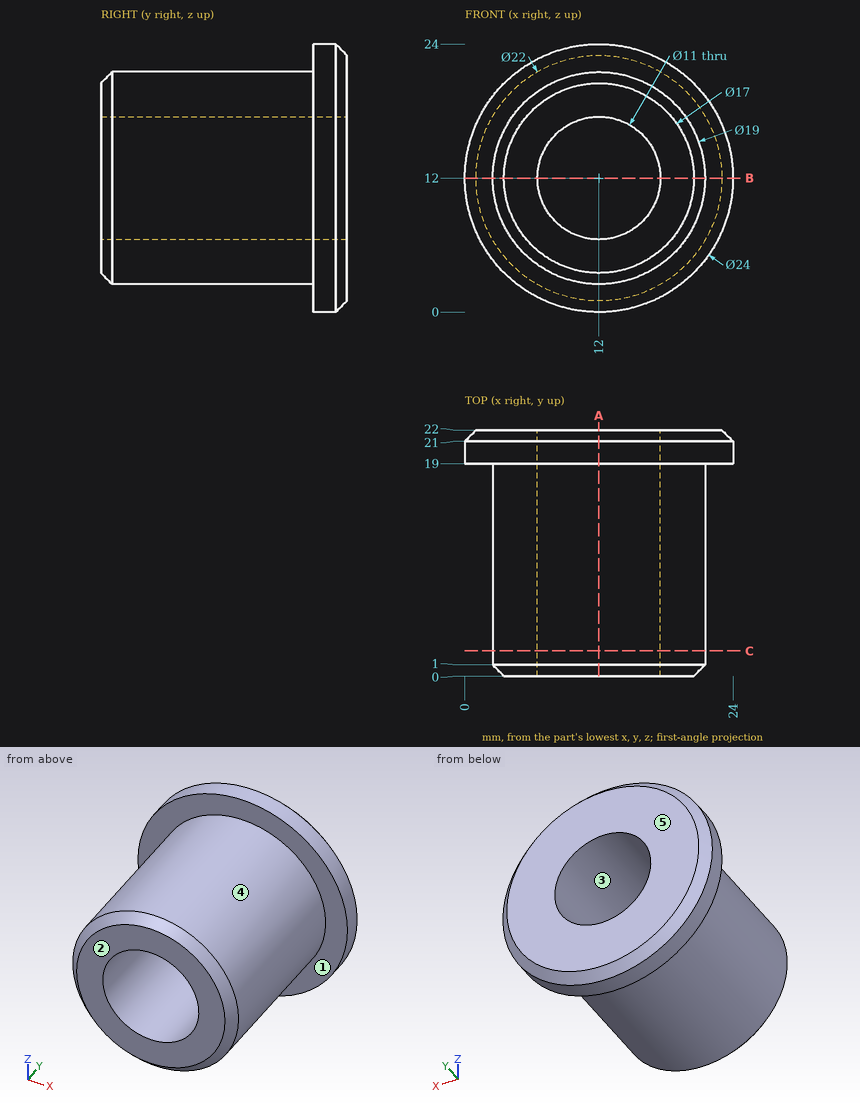
Check sheet for the drawn part. Datum: minimum x, y, z corner. Units: mm. A direction names the side the tool comes from. Give positions to 0.01 mm unless a question says otherwise; leave off trailing zeros. Order: outer loops, then holes, each group sorted by start corner. A loop starts at its lowest first (then second) coordinate and runs counter-clockwise, first axis right, second up.
1. Depth check by flat-ended pin: pin 1 (6.5 mm diameter, centred on x = 12, z = 12, fed in from -Y); pin 2 (5 mm diameter, centred on y = 17.5, z = 12.5, fed in from +X); pin 3 (3 mm diameter, centred on y = 5.5, z = 4.5, fed in from +X); pin 4 (6 mm diameter, centred on x = 14.5, y = 5, fed in from -Z). Enter the tip coordinate at first touch or a pass-through.
Completed:
pin 1: passes through
pin 2: stops at x = 24
pin 3: stops at x = 19.37
pin 4: stops at z = 2.5
2. Draft check along X on the marked faces 3, 4 and 5. Enter one of: pulls with the +X half, pulls with the -X half, needs draft (parallel to the pull), parting line crosses it, or undercut.
Completed:
face 3: undercut
face 4: parting line crosses it
face 5: needs draft
3. Access from +Z, -Z, +X, -X, +Y, -Y to the whole of each face (thin tool, end or side, straight path). Record for the marked faces 1 and 2.
Completed:
face 1: -Y
face 2: +Z, -Z, +X, -X, -Y
4. Scan lines: line 1 (X direction, y = 7.75, z = 12); line 2 (Z direction, x = 16.5, y = 5.5). Record each from-to range of solid material in increasing order.
Completed:
line 1: x = 2.5 to 6.5, 17.5 to 21.5
line 2: z = 3.63 to 8.84, 15.16 to 20.37
5. Sectioned sample at A-A (x = 12). Record the boundary of the cut face in (y, z), then the cut area to 3 significant figures.
Completed:
outline: (0, 3.5) - (1, 2.5) - (19, 2.5) - (19, 0) - (21, 0) - (22, 1) - (22, 6.5) - (0, 6.5) - close; (0, 17.5) - (22, 17.5) - (22, 23) - (21, 24) - (19, 24) - (19, 21.5) - (1, 21.5) - (0, 20.5) - close
area: 189 mm2
6. Sectioned sample at B-B (z = 12). Record the boundary of the cut face in (x, y), then the cut area to 3 significant figures.
Completed:
outline: (0, 19) - (2.5, 19) - (2.5, 1) - (3.5, 0) - (6.5, 0) - (6.5, 22) - (1, 22) - (0, 21) - close; (17.5, 0) - (20.5, 0) - (21.5, 1) - (21.5, 19) - (24, 19) - (24, 21) - (23, 22) - (17.5, 22) - close
area: 189 mm2
7. Sectioned sample at C-C (y = 2.25). Record the boundary of the cut face in (x, z).
Completed:
outline: circle Ø19 at (12, 12); hole circle Ø11 at (12, 12)
